CAD build for the part. Positions are in the model's coordinates, mm. A direction names the side the tool comes from. Coordinates: 2 decimals unless noted, no trailing zeros. Loops run counter-clockwise (first coordinate to the right, second up) from the corner with the lowest first, then second, coordinate; pieces in that order, holes last. Notation, with made-up numbers: (2.5, 81.5) - (46.5, 81.5) arc R8 cw to (46.5, 86.5) - close; hole circle Ø8 at (14.5, -23). An arc over 180 degrees is marked (long way). Put each result on its own line as item: value.
```python
from build123d import *

# Parameters (mm, degrees)
EXTRUDE_1_DEPTH          = 20
SHELL_1_T                = -2
CUT_EXTRUDE_1_DEPTH      = 187
CUT_EXTRUDE_1_DEPTH_BACK = 10
SKETCH_2_R               = 2.75
SKETCH_3_R               = 2.75
CUT_EXTRUDE_2_DEPTH      = 10
SKETCH_4_R               = 2.75
CUT_EXTRUDE_3_DEPTH      = 10


with BuildPart() as part:
    # 草图1 → 凸台-拉伸1 (new body)
    with BuildSketch(Plane.XY):
        with BuildLine():
            Line((0, 0), (609, 0))
            Line((609, 0), (609, 261))
            ThreePointArc((609, 261), (553.322356372, 277.933761371), (516.501351361, 323))
            Line((516.501351361, 323), (316, 323))
            Line((316, 323), (316, 263))
            Line((316, 263), (196, 263))
            Line((196, 263), (196, 323))
            Line((196, 323), (0, 323))
            Line((0, 323), (0, 0))
        make_face()
    extrude(amount=EXTRUDE_1_DEPTH)

    # 抽壳1
    shell_1_openings = [part.faces().sort_by_distance(p)[0] for p in [
        (300.393153284, 153.35137278, 0),
    ]]
    offset(amount=SHELL_1_T, openings=shell_1_openings, kind=Kind.INTERSECTION)

    # 草图2 → 切除-拉伸1 (cut, two sides: drawn at the far end of the back side and taken through both)
    with BuildSketch(Plane.XZ.offset(-321).offset(-CUT_EXTRUDE_1_DEPTH_BACK)):
        with Locations(Location((14, 9, 0), (0, 0, 270))):
            Circle(SKETCH_2_R)
        with Locations(Location((182, 9, 0), (0, 0, 270))):
            Circle(SKETCH_2_R)
        with Locations(Location((98, 9, 0), (0, 0, 270))):
            Circle(SKETCH_2_R)
        with Locations(Location((330, 9, 0), (0, 0, 270))):
            Circle(SKETCH_2_R)
        with Locations(Location((500, 9, 0), (0, 0, 270))):
            Circle(SKETCH_2_R)
        with Locations(Location((415, 9, 0), (0, 0, 270))):
            Circle(SKETCH_2_R)
    extrude(amount=CUT_EXTRUDE_1_DEPTH + CUT_EXTRUDE_1_DEPTH_BACK, mode=Mode.SUBTRACT)

    # 草图3 → 切除-拉伸2 (cut)
    with BuildSketch(Plane.XZ):
        with Locations(Location((14, 9, 0), (0, 0, 270))):
            Circle(SKETCH_3_R)
    extrude(amount=-CUT_EXTRUDE_2_DEPTH, mode=Mode.SUBTRACT)

    # 草图4 → 切除-拉伸3 (cut)
    with BuildSketch(Plane.ZY.offset(-607)):
        with Locations((9, 14)):
            Circle(SKETCH_4_R)
        with Locations((9, 129)):
            Circle(SKETCH_4_R)
        with Locations((9, 244)):
            Circle(SKETCH_4_R)
    extrude(amount=-CUT_EXTRUDE_3_DEPTH, mode=Mode.SUBTRACT)


solid = part.part
```
Q1. Tool access for faces 1 (the flat face through (300, 164, 20)), 2 (the flat face through (196, 293, 10)), 3 (the flat face through (607, 129, 13)): list every direction of +Z, -Z, +X, -X, +Y, -Y with a clear straight run to the whole face (end or side of a thin tool).
Determined:
face 1: +Z, +X, -X, +Y, -Y
face 2: +Z, -Z, +Y
face 3: -Z
Q2. Mould opens along X. For faces 4 (the flat face through (0, 164, 10)), 5 (the cylindrical face through (554.011, 277.476, 9.86)), 6 (the flat face through (257, 261, 9)), 7 (the flat face through (418, 323, 10)) say: +X half, -X half, draft (parallel to the pull), parting line (faces both ways), or undercut.
Determined:
face 4: -X half
face 5: +X half
face 6: undercut
face 7: draft
Q3. Slice it at B-B, the plane y = 285.5. Give the cut face in (x, z).
Determined:
outline: (0, 0) - (2, 0) - (2, 18) - (194, 18) - (194, 0) - (196, 0) - (196, 20) - (0, 20) - close; (316, 0) - (318, 0) - (318, 18) - (540.42, 18) - (540.42, 0) - (543.43, 0) - (543.43, 20) - (316, 20) - close
Q4. Pin check, flat tips, straight feed: pin 1 Ø4.5 at (x, z) = (182, 9) entering from +Y; pin 2 Ø10 at (x, y) = (132.5, 62.5) entering from -Z; pin 3 Ø8 at (y, z) = (51.5, 4.5) entering from -X; pin 4 Ø6 at (x, z) = (238, 11.5) entering from +Y. Stop position of each tip, or through.
Determined:
pin 1: y = 2
pin 2: z = 18
pin 3: x = 0
pin 4: y = 263
Q5. Slice it at C-C, the plane y = 67. Give the cut face in (x, z), then the cut area to 3 significant figures.
Determined:
outline: (0, 0) - (2, 0) - (2, 18) - (607, 18) - (607, 0) - (609, 0) - (609, 20) - (0, 20) - close
area: 1,290 mm2
Q6. Slice it at A-A, the plane x = 221. Give the cut face in (y, z).
Determined:
outline: (0, 0) - (2, 0) - (2, 18) - (261, 18) - (261, 0) - (263, 0) - (263, 20) - (0, 20) - close
Q7. Wall check: L1, parallel to Y at x = 608.35, z = 9; L2, parallel to Y at x = 189, z = 9; L3, parallel to X at y = 166, z = 5.5. Give the ranges that are in metal, low to high. Write a range as from..to.
Determined:
L1: 0..11.25, 16.75..126.25, 131.75..241.25, 246.75..261
L2: 0..2, 321..323
L3: 0..2, 607..609
